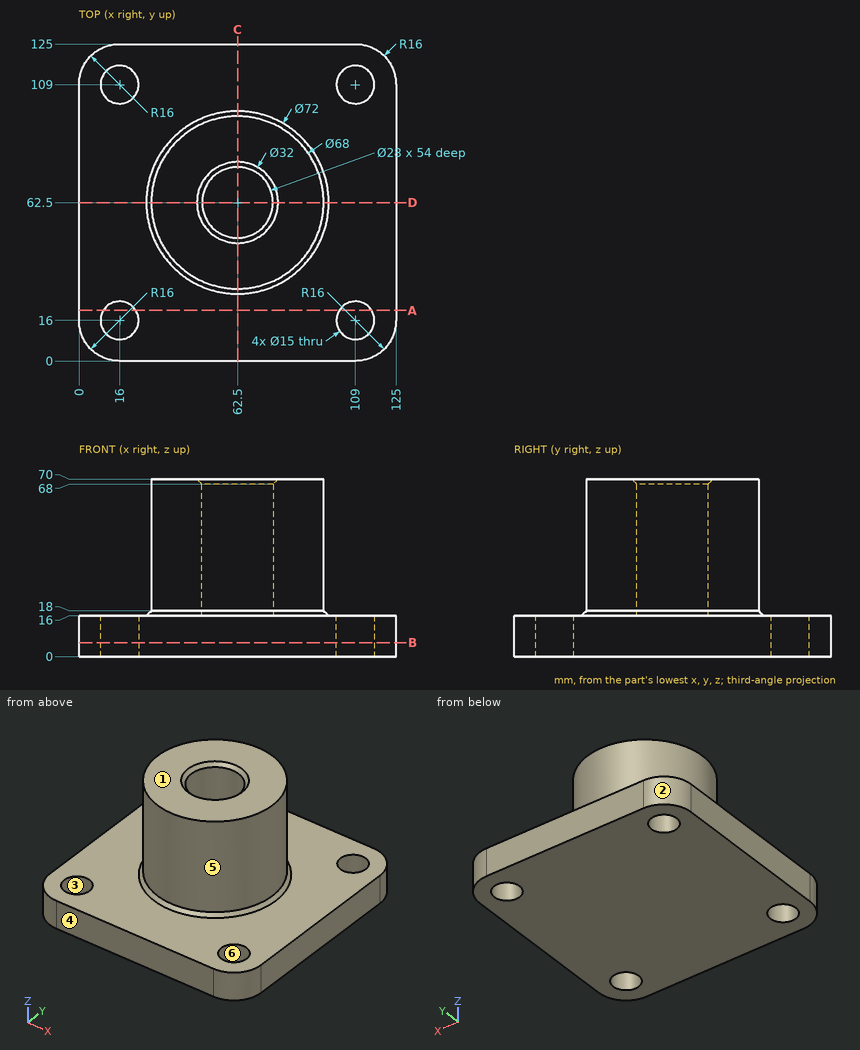
Drawing for the job (mm, zero at the part's lowest x, y, z). A direction names the side the tool comes from. Give positions to 0.01 mm unless a question says otherwise; leave off trailing zeros. Write each loop counter-clockwise with the first axis right and the second up, starting at its lowest first coordinate (ties: lowest second). Pieces come first, ordered by that corner, then holes. Notation, with made-up numbers: (-7, 37.25) -> (31, 37.25) arc R22 ccw to (31, 71.25) -> close; hole circle Ø11 at (26, 88.5). An arc over 180 degrees is marked (long way). Put each result on its own line as item: value. Start each with the question number.
Item 1: Pull direction Y, two halves, no side cores. Call the marked faces 1, 2, 3 and 4: pulls with the +Y half, pulls with the -Y half, needs draft (parallel to the pull), parting line crosses it, or undercut.
Item 2: Pin check, flat tips, straight feed: pin 1 Ø4 at (x, z) = (65.5, 31.5) entering from -Y; pin 2 Ø10 at (y, z) = (67, 31.5) entering from +X; pin 3 Ø2 at (x, z) = (81.5, 28) entering from -Y; pin 4 Ø13.5 at (x, y) = (109, 16) entering from +Z. Stop position of each tip, or through.
Item 3: Wall check: L1, parallel to Y at x = 16, z = 7; L2, parallel to Y at x = 21, z = 15.5; L3, parallel to Z at x = 75, y = 12.5. Give the ranges that are in metal, low to high. Write a range as [from, to].
Item 4: Cut at C-C (x = 62.5). List the corners of the cut face in (y, z).
Item 5: Cut at B-B (z = 5.5). List the corners of the cut face in (x, y), then the cut area to 3 significant figures.
Item 6: Cut at A-A (y = 20). List the corners of the cut face in (x, z), then the cut area to 3 significant figures.
Item 7: Which spindle directions (+Z, -Z, +X, -X, +Y, -Y) get a long thin tool onto all of the face, cutting with end or side? Do the marked faces 5 and 6. Say none if no direction does.
Answer list:
1. face 1: needs draft
1. face 2: pulls with the +Y half
1. face 3: undercut
1. face 4: pulls with the -Y half
2. pin 1: stops at y = 28.51
2. pin 2: stops at x = 96.5
2. pin 3: stops at y = 33.66
2. pin 4: passes through
3. L1: y = [0, 8.5], [23.5, 101.5], [116.5, 125]
3. L2: y = [0, 10.41], [21.59, 103.41], [114.59, 125]
3. L3: z = [0, 16]
4. outline: (0, 0) -> (125, 0) -> (125, 16) -> (98.5, 16) -> (96.5, 18) -> (96.5, 70) -> (78.5, 70) -> (76.5, 68) -> (76.5, 16) -> (48.5, 16) -> (48.5, 68) -> (46.5, 70) -> (28.5, 70) -> (28.5, 18) -> (26.5, 16) -> (0, 16) -> close
5. outline: (0, 16) arc R16 ccw to (16, 0) -> (109, 0) arc R16 ccw to (125, 16) -> (125, 109) arc R16 ccw to (109, 125) -> (16, 125) arc R16 ccw to (0, 109) -> close; hole circle Ø15 at (16, 16); hole circle Ø15 at (16, 109); hole circle Ø15 at (109, 16); hole circle Ø15 at (109, 109)
5. area: 14,700 mm2
6. outline: (0, 0) -> (9.66, 0) -> (9.66, 16) -> (0, 16) -> close; (22.34, 0) -> (102.66, 0) -> (102.66, 16) -> (22.34, 16) -> close; (115.34, 0) -> (125, 0) -> (125, 16) -> (115.34, 16) -> close
6. area: 1,590 mm2
7. face 5: +Z
7. face 6: +Z, -Z
